```python
from build123d import *


with BuildPart() as part:
    # Pawn Profile Sketch → Pawn Body Revolve (revolve)
    with BuildSketch(Plane.XY, mode=Mode.PRIVATE) as pawn_body_revolve_sk:
        with BuildLine():
            Line((0, 0), (15, 0))
            Line((15, 0), (15, 3))
            Line((15, 3), (13, 5))
            ThreePointArc((13, 5), (13.688325627, 10.216881481), (10, 13.97))
            Line((10, 13.97), (10, 14.97))
            ThreePointArc((10, 14.97), (9.414213562, 16.384213562), (8, 16.97))
            ThreePointArc((8, 16.97), (5.019495729, 28.81539847), (5, 41.03))
            ThreePointArc((5, 41.03), (6.412519214, 42.380086131), (6, 44.29))
            ThreePointArc((6, 44.29), (9, 54.436534055), (0, 60))
            Line((0, 60), (0, 0))
        make_face()
    revolve(pawn_body_revolve_sk.sketch.rotate(Axis((0, 0, 0), (0, 1, 0)), 90), axis=Axis((0, 0, 0), (0, 1, 0)))


solid = part.part
```
CAD build for the part. Positions are in the model's coordinates, mm. A direction names the side the tool comes from. Coordinates: 2 decimals unless noted, no trailing zeros. Write each loop counter-clockwise with the first axis right and the second up, starting at its lowest first coordinate (ties: lowest second). Pieces come first, ordered by that corner, then holes. Notation, with made-up numbers: (48.25, 51) -> (91.25, 51) arc R19 ccw to (91.25, 68) -> close; hole circle Ø8 at (-23.5, -2). An arc over 180 degrees is marked (long way). Return JSON: item names as keys, results as strings. Group by question number.
Q1. Drill centre lines: line 1 (Y direction, x = -8, z = 2.5); line 2 (Z direction, x = 0.5, y = 16); line 3 (Z direction, x = -5.5, y = 43.5). Where is each one in solid material? Low to high.
Q2. Which spindle directions (+Z, -Z, +X, -X, +Y, -Y) get a long thin tool onto all of the face, cutting with end or side? Do faces 1 (the face through (-0.44, 14.48, 9.99)), 2 (the face through (-12.65, 1.52, -8.06)). Say none if no direction does.
Q3. Cut at A-A, the plane y = 32. Give the cut face in (x, z).
Q4. Flat gauge pins, fed straight in: pin 1 (1.5 mm diameter, centred on x = -5, y = 33, fed in from +Z); pin 2 (1.5 mm diameter, centred on y = 40.5, z = -1, fed in from -X); pin 3 (10 mm diameter, centred on x = -6, y = 43, fed in from -Z). Where does each tip first touch, or does it go through?
Returned:
{
 "1": {"line 1": "y = 0 to 16.93, 46.93 to 55.73", "line 2": "z = -9.7 to 9.7", "line 3": "z = -3.33 to 3.33"},
 "2": {"face 1": "+Y", "face 2": "+Y, -Y"},
 "3": {"outline": "circle Ø9.45 at (0, 0)"},
 "4": {"pin 1": "stops at z = 1.95", "pin 2": "stops at x = -5.44", "pin 3": "stops at z = -7.88"}
}
